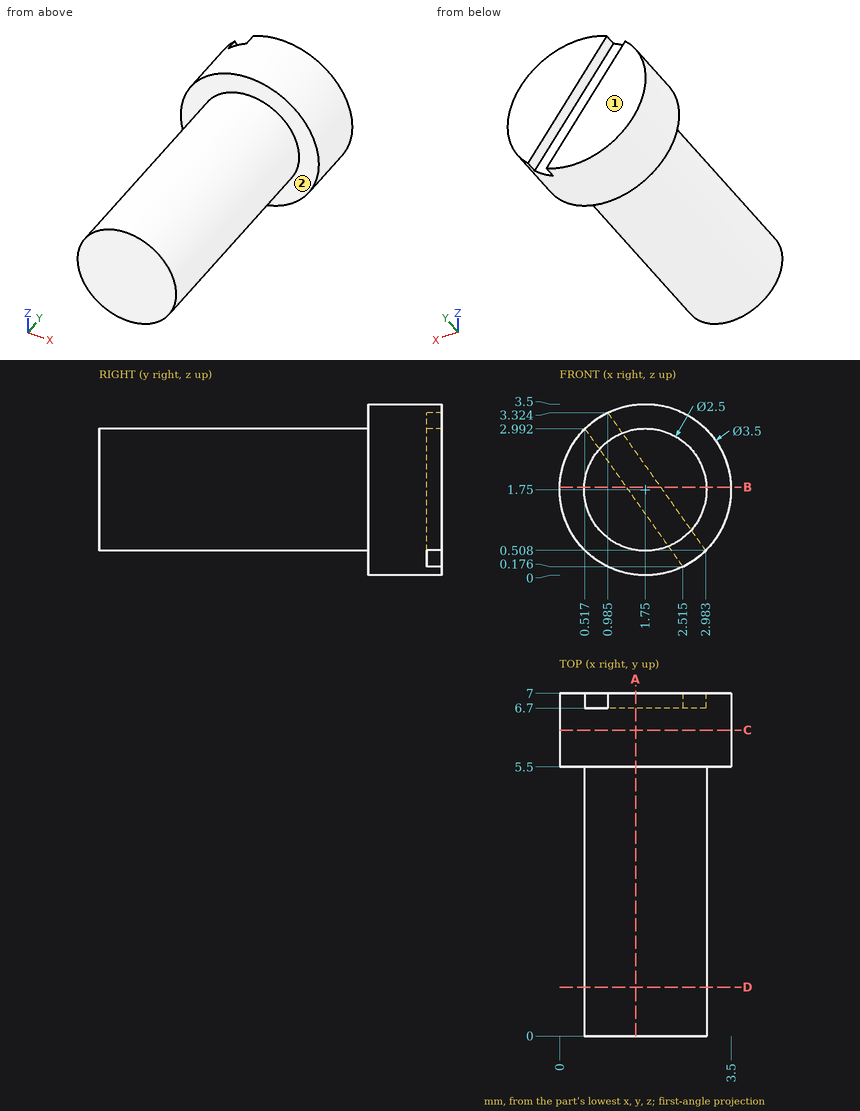
Study the drawing (mm; zero at the part's minimum x, y, z) and answer. A direction names the side the tool comes from. Round coordinates to 2 decimals unless told otherwise and drop trailing zeros. Write each loop counter-clockwise with the first axis right and the second up, starting at its lowest first coordinate (ties: lowest second). Pieces come first, ordered by that corner, then holes. Notation, with made-up numbers: (19, -15) - (67, -15) arc R30 cw to (67, 15) - close; hole circle Ø2 at (4, 53.5). An arc over 180 degrees is marked (long way). Return JSON: item names as keys, results as strings. Group by question number.
Q1. Find the intervals of material crossed by L1, parallel to Z at x = 1.55, y = 1.5; L2, parallel to Y at x = 2.95, z = 1.2; L3, parallel to Y at x = 1.05, z = 3.05, in increasing order.
Q2. The part is cut by section A-A on x = 1.55. Write down the section's boundary in (y, z), then the cut area to 3 significant figures.
Q3. The part is cut by section D-D on y = 1. Write down the section's boundary in (x, z).
Q4. Each of these flat-tipped pins is pushed along its axis until it touches: pin 1 Ø2 at (x, y) = (2, 5.5) entering from +Z; pin 2 Ø2 at (x, y) = (1, 0.5) entering from -Z. Where does it stop, or does it pass through?
Q5. The part is cut by section B-B on z = 1.8. Write down the section's boundary in (x, y).
Q6. For the marked faces 1 and 2, determine the directions among +Z, -Z, +X, -X, +Y, -Y from which every point of the face is accessible in a straight line to the end or side of a thin tool.
Q7. The part is cut by section C-C on y = 6.25. Write down the section's boundary in (x, z).
Solved:
{
 "1": {"L1": "0.52 to 2.98", "L2": "5.5 to 7", "L3": "5.5 to 6.7"},
 "2": {"outline": "(0, 0.52) - (5.5, 0.52) - (5.5, 0.01) - (7, 0.01) - (7, 1.54) - (6.7, 1.54) - (6.7, 2.53) - (7, 2.53) - (7, 3.49) - (5.5, 3.49) - (5.5, 2.98) - (0, 2.98) - close", "area": "18.5 mm²"},
 "3": {"outline": "circle Ø2.5 at (1.75, 1.75)"},
 "4": {"pin 1": "z = 3.5", "pin 2": "z = 0.5"},
 "5": {"outline": "(0, 5.5) - (0.5, 5.5) - (0.5, 0) - (3, 0) - (3, 5.5) - (3.5, 5.5) - (3.5, 7) - (2.07, 7) - (2.07, 6.7) - (1.36, 6.7) - (1.36, 7) - (0, 7) - close"},
 "6": {"face 1": "+Z, -Z, +X, -X, +Y", "face 2": "-Y"},
 "7": {"outline": "circle Ø3.5 at (1.75, 1.75)"}
}
